Here's the drawing with two shaded views (mm, measured from the low corner). I have some questions. Coordinates: 2 decimals unless noted, no trailing zeros. Write each loop counter-clockwise with the first axis right and the second up, starting at its lowest first coordinate (ties: lowest second). Pieces come first, ordered by that corner, then holes.
Item 1: If I drill on line 1 (X direction, y = 0.5, z = 20.5); line 2 (Z direction, x = 2.25, y = 0.55); line 3 (Y direction, x = 9.5, z = 9.75), over which ranges is the centre line in solid material (lowest first)?
Item 2: If we section it at B-B (x = 7.9): Please give me the cut outline in (y, z).
Item 3: If we section it at A-A (z = 4.5): Please give me the cut outline in (x, y).
Item 4: I'm going to push flat-ended pins straight in: pin 1 Ø4 at (x, z) = (10.5, 16.5) entering from +Y; pin 2 Ø1.9 at (x, y) = (2.5, 2.5) entering from -Z; pin 3 Ø0.6 at (y, z) = (0.5, 21.5) entering from -X. Where does each tip first touch, or does it pass through?
Item 5: If we section it at C-C (y = 1.9): Please give me the cut outline in (x, z), then the cut area to 3 significant figures.
Item 6: If we section it at D-D (z = 14.75): Please give me the cut outline in (x, y).
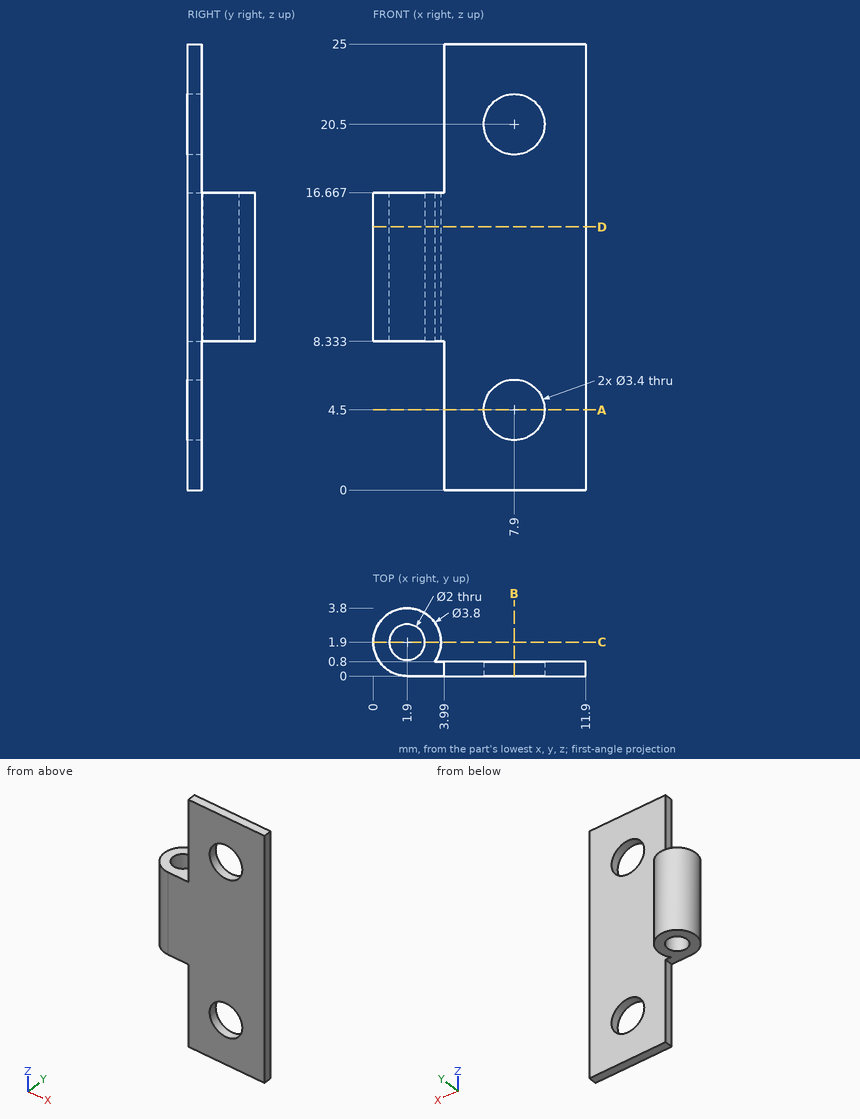
Answer list:
1. line 1: x = 3.99 to 6.2, 9.6 to 11.9
1. line 2: z = 8.33 to 16.67
1. line 3: y = 0 to 0.8
2. outline: (0, 0) - (0.8, 0) - (0.8, 2.8) - (0, 2.8) - close; (0, 6.2) - (0.8, 6.2) - (0.8, 18.8) - (0, 18.8) - close; (0, 22.2) - (0.8, 22.2) - (0.8, 25) - (0, 25) - close
3. outline: (3.99, 0) - (6.2, 0) - (6.2, 0.8) - (3.99, 0.8) - close; (9.6, 0) - (11.9, 0) - (11.9, 0.8) - (9.6, 0.8) - close
4. pin 1: stops at y = 0.8
4. pin 2: stops at z = 8.33
4. pin 3: stops at x = 3.99
5. outline: (0, 8.33) - (0.9, 8.33) - (0.9, 16.67) - (0, 16.67) - close; (2.9, 8.33) - (3.8, 8.33) - (3.8, 16.67) - (2.9, 16.67) - close
5. area: 15.0 mm2
6. outline: (1.9, 0) - (11.9, 0) - (11.9, 0.8) - (3.45, 0.8) arc R1.9 ccw (long way) to start; hole circle Ø2 at (1.9, 1.9)
